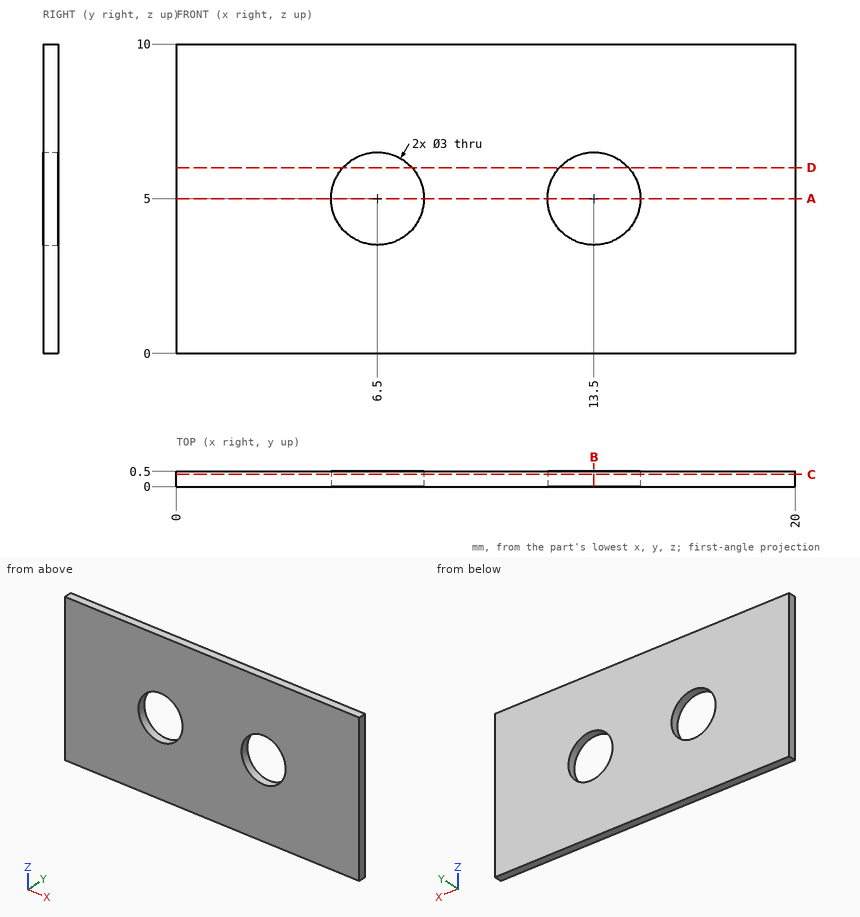
Could you check a few things on this drawing? It's one solid part, dimensions in mm from its lowest x, y, z. Round coordinates to 2 decimals unless told otherwise and drop trailing zeros. Loops run counter-clockwise (first coordinate to the right, second up) from the corner with the lowest first, then second, coordinate; pieces in that order, holes last. Notation, with made-up numbers: (14.25, 9) -> (65.25, 9) arc R30 cw to (65.25, 41) -> close; hole circle Ø2 at (85.25, -16.75). An arc over 180 degrees is marked (long way). Answer as CSV lines item,"result".
1. If we section it at D-D on z = 6: Please give me the cut outline in (x, y).
Final values:
outline,"(0, 0) -> (5.38, 0) -> (5.38, 0.5) -> (0, 0.5) -> close; (7.62, 0) -> (12.38, 0) -> (12.38, 0.5) -> (7.62, 0.5) -> close; (14.62, 0) -> (20, 0) -> (20, 0.5) -> (14.62, 0.5) -> close"
2. If we section it at C-C on y = 0.4: Please give me the cut outline in (x, z), plus the area to 3 significant figures.
Final values:
outline,"(0, 0) -> (20, 0) -> (20, 10) -> (0, 10) -> close; hole circle Ø3 at (6.5, 5); hole circle Ø3 at (13.5, 5)"
area,"186 mm^2"
3. If we section it at B-B on x = 13.5: Please give me the cut outline in (y, z), plus the area to 3 significant figures.
Final values:
outline,"(0, 0) -> (0.5, 0) -> (0.5, 3.5) -> (0, 3.5) -> close; (0, 6.5) -> (0.5, 6.5) -> (0.5, 10) -> (0, 10) -> close"
area,"3.50 mm^2"
4. If I drill on L1, parallel to X at y = 0.25, z = 5; L2, parallel to Z at x = 13.5, y = 0.3; L3, parallel to X at y = 0.1, z = 3.75, over which ranges is the centre line in solid material (lowest first)?
Final values:
L1,"x = 0 to 5, 8 to 12, 15 to 20"
L2,"z = 0 to 3.5, 6.5 to 10"
L3,"x = 0 to 5.67, 7.33 to 12.67, 14.33 to 20"
5. If we section it at A-A on z = 5: Please give me the cut outline in (x, y), plus the area to 3 significant figures.
Final values:
outline,"(0, 0) -> (5, 0) -> (5, 0.5) -> (0, 0.5) -> close; (8, 0) -> (12, 0) -> (12, 0.5) -> (8, 0.5) -> close; (15, 0) -> (20, 0) -> (20, 0.5) -> (15, 0.5) -> close"
area,"7.00 mm^2"
